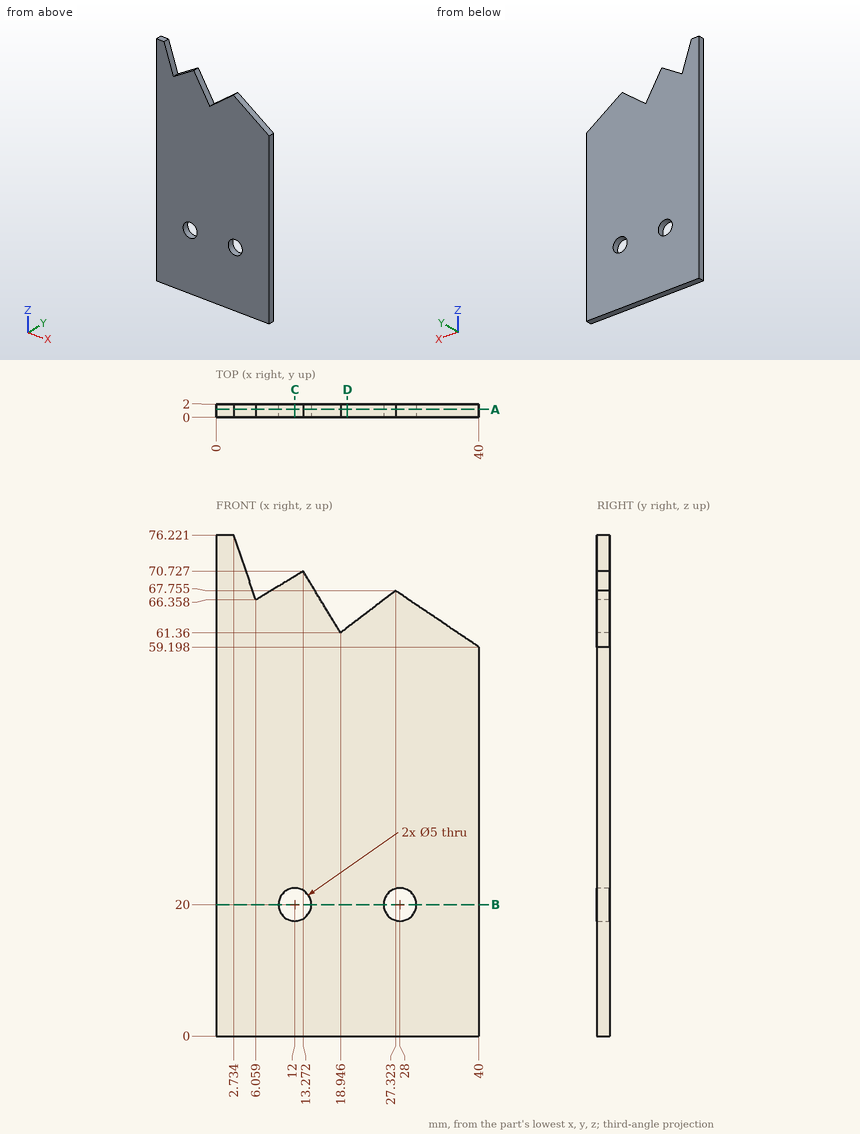
Drawing for the job (mm, zero at the part's lowest x, y, z). Round coordinates to 2 decimals unless told otherwise and drop trailing zeros. Write each loop counter-clockwise with the first axis right and the second up, starting at its lowest first coordinate (ties: lowest second). Pieces come first, ordered by that corner, then holes. Notation, with made-up numbers: M 38,61 L 64,61 A16 ccw 64,67 Z; hole C 64,46.5 d8. An arc over 180 degrees is marked long. One line per question, with ' | ' between items.
1. Cut at D-D on x = 20. Write the cut outline in (y, z) (1 decimal).
Working result:
outline: M 0,0 L 2,0 L 2,62.2 L 0,62.2 Z
2. Probe L1, parallel to X at y = 1, z = 20; L2, parallel to Z at x = 12.5, y = 0.65; L3, parallel to Z at x = 28.5, y = 0.6. List the from-to ranges inside material, lowest first. Write a range as from..to.
Working result:
L1: 0..9.5, 14.5..25.5, 30.5..40 | L2: 0..17.55, 22.45..70.26 | L3: 0..17.55, 22.45..66.96
3. Cut at B-B on z = 20. Write the cut outline in (x, y).
Working result:
outline: M 0,0 L 9.5,0 L 9.5,2 L 0,2 Z; M 14.5,0 L 25.5,0 L 25.5,2 L 14.5,2 Z; M 30.5,0 L 40,0 L 40,2 L 30.5,2 Z
4. Cut at A-A on y = 1.2. Write the cut outline in (x, z) (1 decimal), and give its area (3 significant figures).
Working result:
outline: M 0,0 L 40,0 L 40,59.2 L 27.3,67.8 L 18.9,61.4 L 13.3,70.7 L 6.1,66.4 L 2.7,76.2 L 0,76.2 Z; hole C 12,20 d5; hole C 28,20 d5 | area: 2,620 mm2
5. Cut at C-C on x = 12. Write the cut outline in (y, z), and give its area (3 significant figures).
Working result:
outline: M 0,0 L 2,0 L 2,17.5 L 0,17.5 Z; M 0,22.5 L 2,22.5 L 2,69.96 L 0,69.96 Z | area: 130 mm2
